from build123d import *

# Parameters (mm, degrees)
SKETCH1_R             = 75
BOSS_EXTRUDE1_DEPTH   = 18
SKETCH2_R             = 24
CUT_EXTRUDE1_DEPTH    = 12
SKETCH5_R             = 24
SKETCH6_R             = 65
BOSS_EXTRUDE2_DEPTH   = 170
F_14_0_14_HOLE1_D     = 14
F_14_0_14_HOLE1_DEPTH = 18
CIRPATTERN1_COUNT     = 4
SKETCH10_R            = 29
BOSS_EXTRUDE3_DEPTH   = 70
SKETCH11_R            = 19
CUT_EXTRUDE2_DEPTH    = 187
SKETCH13_R            = 12.5
CUT_EXTRUDE3_START    = -25
SKETCH14_R            = 65
SKETCH14_R_2          = 55
CUT_EXTRUDE3_DEPTH    = 25
SKETCH15_R            = 24
CUT_EXTRUDE4_DEPTH    = 60
SKETCH16_W            = 32
SKETCH16_H            = 71.063102747
BOSS_EXTRUDE4_DEPTH   = 12.5
SKETCH17_R            = 8
CUT_EXTRUDE5_DEPTH    = 25


with BuildPart() as part:
    # Sketch1 → Boss-Extrude1 (new body)
    with BuildSketch(Plane.XY):
        Circle(SKETCH1_R)
    extrude(amount=BOSS_EXTRUDE1_DEPTH)

    # Sketch2 → Cut-Extrude1 (cut)
    with BuildSketch(Plane.XY.offset(18)):
        Circle(SKETCH2_R)
    extrude(amount=-CUT_EXTRUDE1_DEPTH, mode=Mode.SUBTRACT)

    # Sweep1: sweep along a path in Sketch3
    with BuildLine(Plane(origin=(0, 0, 0), x_dir=(0, 0, -1), z_dir=(1, 0, 0))) as sweep1_path:
        Line((12, 0), (-239, 0))
        ThreePointArc((-239, 0), (-267.284271247, -11.715728753), (-279, -40))
        Line((-279, -40), (-279, -43))
    # Sketch5 → Sweep1 (sweep)
    with BuildSketch(Plane(origin=(0, 0, -12), x_dir=(-1, 0, 0), z_dir=(0, 0, -1))):
        Circle(SKETCH5_R)
    sweep(path=sweep1_path.line)

    # Sketch6 → Boss-Extrude2 (add)
    with BuildSketch(Plane(origin=(0, 0, 57), x_dir=(-1, 0, 0), z_dir=(0, 0, -1))):
        Circle(SKETCH6_R)
    extrude(amount=-BOSS_EXTRUDE2_DEPTH)

    # Ø14.0 (14) Hole1
    with Locations(Plane(origin=(0, 0, 0), x_dir=(-1, 0, 0), z_dir=(0, 0, -1))):
        with Locations((-38.905866791, 38.905866791)):
            f_14_0_14_hole1 = Hole(F_14_0_14_HOLE1_D / 2, depth=F_14_0_14_HOLE1_DEPTH)

    # CirPattern1: Ø14.0 (14) Hole1 ×4 about axis
    cirpattern1_axis = Axis((0, 0, 0), (0, 0, 1))
    for i in range(1, CIRPATTERN1_COUNT):
        add(f_14_0_14_hole1.rotate(cirpattern1_axis, i * 360 / CIRPATTERN1_COUNT), mode=Mode.SUBTRACT)

    # Sketch10 → Boss-Extrude3 (add)
    with BuildSketch(Plane(origin=(0, 0, 0), x_dir=(1, 0, 0), z_dir=(0, 1, 0))):
        with Locations(Location((0, -171.843858555, 0), (0, 0, 270))):
            Circle(SKETCH10_R)
    extrude(amount=-BOSS_EXTRUDE3_DEPTH)

    # Sketch11 → Cut-Extrude2 (cut)
    with BuildSketch(Plane(origin=(0, 0, -12), x_dir=(-1, 0, 0), z_dir=(0, 0, -1))):
        Circle(SKETCH11_R)
    extrude(amount=-CUT_EXTRUDE2_DEPTH, mode=Mode.SUBTRACT)

    # Cut-Sweep1: sweep along a path in Sketch12
    with BuildLine(Plane(origin=(0, 0, 0), x_dir=(0, 0, -1), z_dir=(1, 0, 0))) as cut_sweep1_path:
        Line((-279, -43), (-279, -30))
        ThreePointArc((-279, -30), (-270.213203436, -8.786796564), (-249, 0))
        Line((-249, 0), (-239, 0))
    # Sketch13 → Cut-Sweep1 (sweep, cut)
    with BuildSketch(Plane.XZ.offset(43)):
        with Locations((0, 279)):
            Circle(SKETCH13_R)
    sweep(path=cut_sweep1_path.line, mode=Mode.SUBTRACT)

    # Sketch14 → Cut-Extrude3 (cut)
    with BuildSketch(Plane.XY.offset(227).offset(CUT_EXTRUDE3_START)):
        with Locations(Location((0, 0, 0), (0, 0, 180))):
            Circle(SKETCH14_R)
        Circle(SKETCH14_R_2, mode=Mode.SUBTRACT)
    extrude(amount=CUT_EXTRUDE3_DEPTH, mode=Mode.SUBTRACT)

    # Sketch15 → Cut-Extrude4 (cut)
    with BuildSketch(Plane(origin=(0, -70, 0), x_dir=(-1, 0, 0), z_dir=(0, -1, 0))):
        with Locations(Location((0, -171.843858555, 0), (0, 0, 90))):
            Circle(SKETCH15_R)
    extrude(amount=-CUT_EXTRUDE4_DEPTH, mode=Mode.SUBTRACT)

    # Sketch16 → Boss-Extrude4 (add, symmetric)
    with BuildSketch(Plane(origin=(0, 0, 0), x_dir=(0, 0, -1), z_dir=(1, 0, 0))):
        with Locations((-129, 59.468448626)):
            Rectangle(SKETCH16_W, SKETCH16_H)
    extrude(amount=BOSS_EXTRUDE4_DEPTH, both=True)

    # Sketch17 → Cut-Extrude5 (cut)
    with BuildSketch(Plane(origin=(12.5, 0, 0), x_dir=(0, 0, -1), z_dir=(1, 0, 0))):
        with Locations((-129, 78)):
            Circle(SKETCH17_R)
    extrude(amount=-CUT_EXTRUDE5_DEPTH, mode=Mode.SUBTRACT)


solid = part.part
CAD build for the part. Positions are in the model's coordinates, mm. A direction names the side the tool comes from. Coordinates: 2 decimals unless noted, no trailing zeros. Write each loop counter-clockwise with the first axis right and the second up, starting at its lowest first coordinate (ties: lowest second). Pieces come first, ordered by that corner, then holes. Notation, with made-up numbers: M -17,77.5 L -2,77.5 A15 ccw -2,104.5 Z; hole C 47.5,31.25 d4. An arc over 180 degrees is marked long. Answer as a JSON object with one key per item and string values. Group by question number.
1) Saw through at B-B (x = 0). Give the number of separate pieces and of enclosed holes in the cut face, plus the area to 3 significant figures.
2) Wall check: line 1 (Y direction, x = 0, z = 129); line 2 (Z direction, x = 31.5, y = 42.5); line 3 (X direction, y = 1, z = 70). Give the ranges that are in metal, low to high. Write a range as from..to.
3) Tool access for faces 5 (the face through (-17.646, -65.269, 148.83)), 6 (the face through (22, -70, 161)), 7 (the face through (0, 5, 175)): list every direction of +Z, -Z, +X, -X, +Y, -Y with a clear straight run to the whole face (end or side of a thin tool).
4) Saw through at A-A (z = 129). Write the cut outline in (x, y), plus the area to 3 significant figures.
5) Mould opens along Y. For faces 1 (the face through (0.18, 80.4, 121.37)), 2 (the face through (23.977, -1.055, 37.773)), 3 (the face through (-18, 7, -12)), 4 (the face through (11.923, -3.755, 243.93)) say: +Y half, -Y half, draft (parallel to the pull), parting line (faces both ways), or undercut.
6) Saw through at C-C (z = 35). Write the cut outline in (x, y).
7) Saw through at D-D (z = 165). Write the cut outline in (x, y), plus the area to 3 significant figures.
8) Pin check, flat tips, straight feed: pin 1 Ø16 at (x, y) = (38.91, -38.91) entering from -Z; pin 2 Ø7.5 at (x, y) = (1.5, -5) entering from +Z; pin 3 Ø12 at (y, z) = (53.5, 129.5) entering from -X; pin 4 Ø9.5 at (y, z) = (78, 129) entering from -X (3 decimals). Stop position of each tip, or through.
Values follow:
{
 "1": {"separate pieces": "2", "enclosed holes": "1", "area": "20,000 mm2"},
 "2": {"line 1": "y = -65..-19, 19..70, 86..95", "line 2": "z = 0..18, 57..227", "line 3": "x = -64.99..-18.97, 18.97..64.99"},
 "3": {"face 5": "-Y", "face 6": "+Z, +X, -X, -Y", "face 7": "-Z"},
 "4": {"outline": "M -12.5,63.79 A65 ccw long 12.5,63.79 L 12.5,70 L -12.5,70 Z; M -12.5,86 L 12.5,86 L 12.5,95 L -12.5,95 Z; hole C 0,0 d38", "area": "12,500 mm2"},
 "5": {"face 1": "undercut", "face 2": "parting line", "face 3": "draft", "face 4": "undercut"},
 "6": {"outline": "C 0,0 d48; hole C 0,0 d38"},
 "7": {"outline": "M -28.18,-70 L -23,-70 L -23,-10 L -16.16,-10 A19 cw long 16.16,-10 L 23,-10 L 23,-70 L 28.18,-70 L 28.18,-58.57 A65 ccw long -28.18,-58.57 Z", "area": "9,980 mm2"},
 "8": {"pin 1": "stops at z = 0", "pin 2": "stops at z = 294.81", "pin 3": "stops at x = -44.37", "pin 4": "passes through"}
}
